Source: three-view drawing plus pictorial views. Frame: mm from the lowest corner of the part. Round coordinates to 2 decimals unless told otherwise and drop trailing zeros. Loops run counter-clockwise (first coordinate to the right, second up) from the corner with the lowest first, then second, coordinate; pieces in that order, holes last. Notation, with made-up numbers: (81.25, 81.25) -> (88.25, 81.25) arc R21 cw to (88.25, 91.25) -> close; hole circle Ø7 at (-24, 13). An arc over 180 degrees is marked (long way). Put each result on its own line as item: value. Start each with the question number.
1. Cut plane A-A (z = 4). Return the cut outline in (x, y).
2. Material intervals for L1, parallel to Y at x = 25, z = 2.75; L2, parallel to X at y = 22, z = 3.25; L3, parallel to X at y = 20, z = 0.55, sorted ascending.
3. Cut plane B-B (y = 25). Return the cut outline in (x, z).
4. Cut plane C-C (x = 105). Return the cut outline in (y, z), then the cut area to 4 significant figures.
5. Contact query for a flat-ended pin moving along its axis: pin 1 (4 mm diameter, centred on x = 83, y = 40, fed in from -Z). Output: stop coordinate, or through.
6. Cut plane D-D (x = 27). Return the cut outline in (y, z), then the cut area to 3 significant figures.
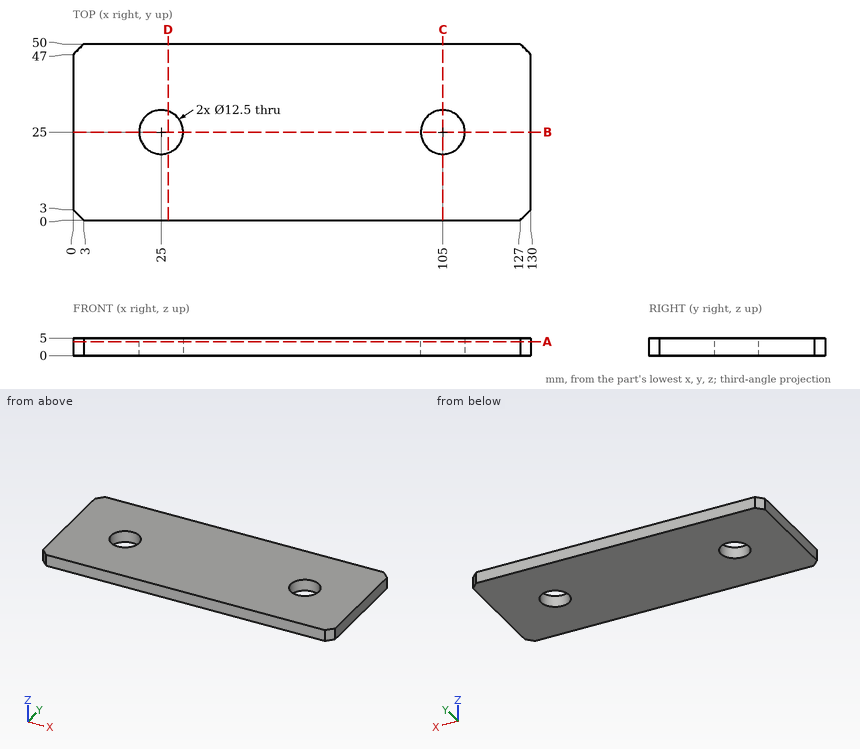
Solution:
1. outline: (0, 3) -> (3, 0) -> (127, 0) -> (130, 3) -> (130, 47) -> (127, 50) -> (3, 50) -> (0, 47) -> close; hole circle Ø12.5 at (25, 25); hole circle Ø12.5 at (105, 25)
2. L1: y = 0 to 18.75, 31.25 to 50
2. L2: x = 0 to 19.52, 30.48 to 99.52, 110.48 to 130
2. L3: x = 0 to 21.25, 28.75 to 101.25, 108.75 to 130
3. outline: (0, 0) -> (18.75, 0) -> (18.75, 5) -> (0, 5) -> close; (31.25, 0) -> (98.75, 0) -> (98.75, 5) -> (31.25, 5) -> close; (111.25, 0) -> (130, 0) -> (130, 5) -> (111.25, 5) -> close
4. outline: (0, 0) -> (18.75, 0) -> (18.75, 5) -> (0, 5) -> close; (31.25, 0) -> (50, 0) -> (50, 5) -> (31.25, 5) -> close
4. area: 187.5 mm^2
5. pin 1: stops at z = 0
6. outline: (0, 0) -> (19.08, 0) -> (19.08, 5) -> (0, 5) -> close; (30.92, 0) -> (50, 0) -> (50, 5) -> (30.92, 5) -> close
6. area: 191 mm^2
